```python
from build123d import *

# Parameters (mm, degrees)
SKETCH1_R           = 25
SKETCH1_R_2         = 24
BOSS_EXTRUDE1_DEPTH = 1590
SKETCH4_R           = 30
BOSS_EXTRUDE2_DEPTH = 5
BOSS_EXTRUDE3_START = 5
SKETCH5_R           = 30
BOSS_EXTRUDE3_DEPTH = 5


with BuildPart() as part:
    # Sketch1 → Boss-Extrude1 (new body)
    with BuildSketch(Plane.XY):
        Circle(SKETCH1_R)
        Circle(SKETCH1_R_2, mode=Mode.SUBTRACT)
    extrude(amount=BOSS_EXTRUDE1_DEPTH)

    # Sketch4 → Boss-Extrude2 (add)
    with BuildSketch(Plane(origin=(0, 0, 0), x_dir=(-1, 0, 0), z_dir=(0, 0, -1))):
        Circle(SKETCH4_R)
    extrude(amount=BOSS_EXTRUDE2_DEPTH)

    # Sketch5 → Boss-Extrude3 (add)
    with BuildSketch(Plane.XY.offset(1590).offset(BOSS_EXTRUDE3_START)):
        with Locations(Location((0, 0, 0), (0, 0, 180))):
            Circle(SKETCH5_R)
    extrude(amount=-BOSS_EXTRUDE3_DEPTH)


solid = part.part
```
Here's how the part is built. I have some questions about the finished solid (model axes, mm). A direction names the side the tool comes from. Coordinates: 2 decimals unless noted, no trailing zeros. Order: outer loops, then holes, each group sorted by start corner. A loop starts at its lowest first (then second) coordinate and runs counter-clockwise, first axis right, second up. Notation, with made-up numbers: (-9, -2) - (44, -2) arc R14 ccw to (44, 24) - close; hole circle Ø8 at (68, 11). An arc over 180 degrees is marked (long way). One line per question, with ' | ' between items.
(1) Will these pins go through, and if not, where does the flat tip stop? pin 1 (4 mm diameter, centred on x = 6.5, z = 603, fed in from +Y); pin 2 (10 mm diameter, centred on x = -12.5, z = 967, fed in from +Y); pin 3 (5 mm diameter, centred on x = 0, z = 969, fed in from +Y).
Report:
pin 1: stops at y = 24.59 | pin 2: stops at y = 23.85 | pin 3: stops at y = 25
(2) Suppose I cut it at A-A on y = 0. List the corners of the cut face in (x, z) for me, and give its area (3 significant figures).
Report:
outline: (-30, -5) - (30, -5) - (30, 0) - (25, 0) - (25, 1590) - (30, 1590) - (30, 1595) - (-30, 1595) - (-30, 1590) - (-25, 1590) - (-25, 0) - (-30, 0) - close; hole (-24, 0) - (24, 0) - (24, 1590) - (-24, 1590) - close | area: 3,780 mm2
(3) If I drill on L1, parallel to Y at x = 0, z = 694.5; L2, parallel to Z at x = -18, y = -22.5; L3, parallel to X at y = 1, z = 676, over which ranges is the centre line in solid material (lowest first)?
Report:
L1: y = -25 to -24, 24 to 25 | L2: z = -5 to 0, 1590 to 1595 | L3: x = -24.98 to -23.98, 23.98 to 24.98
(4) For faces 5 (the cylindrical face through (-16.128, -25.296, 1592.535)), 6 (the flat face through (0, 0, 0)), which set-ups out of +Z, -Z, +X, -X, +Y, -Y let a thin tool reach every point of the face, with its end or its side?
Report:
face 5: +Z, -Z | face 6: none
(5) Suppose I cut it at C-C on z = 1086. List the corners of the cut face in (x, y) for me.
Report:
outline: circle Ø50 at (0, 0); hole circle Ø48 at (0, 0)
(6) If we mould it in two halves opening along Z, with no side actions, what happens to faces 1 (the flat face through (0, 0, -5)), 2 (the flat face through (7, -25, 1590)), 3 (the cylindrical face through (29.97, 1.32, -2.46)), 4 (the flat face through (0, 0, 1595))? For each: pulls with the +Z half, pulls with the -Z half, needs draft (parallel to the pull), parting line crosses it, or undercut.
Report:
face 1: pulls with the -Z half | face 2: undercut | face 3: needs draft | face 4: pulls with the +Z half
